from build123d import *

# Parameters (mm, degrees)
SKETCH_1_R      = 17.5
EXTRUDE_1_DEPTH = 57
SKETCH_2_R      = 23
EXTRUDE_2_DEPTH = 84
SKETCH_3_R      = 17
EXTRUDE_3_DEPTH = 6
SKETCH_4_R      = 13
EXTRUDE_4_DEPTH = 43
CHAMFER_1_SIZE  = 0.5


with BuildPart() as part:
    # 草图1 → 凸台-拉伸1 (new, symmetric)
    with BuildSketch(Plane.XY):
        with Locations(Location((0, 0, 0), (0, 0, 180))):
            Circle(SKETCH_1_R)
    extrude(amount=EXTRUDE_1_DEPTH, both=True)

    # 草图2 → 凸台-拉伸2 (add)
    with BuildSketch(Plane(origin=(0, 0, -57), x_dir=(-1, 0, 0), z_dir=(0, 0, -1))):
        with Locations(Location((0, 0, 0), (0, 0, 180))):
            Circle(SKETCH_2_R)
    extrude(amount=EXTRUDE_2_DEPTH)

    # 草图3 → 凸台-拉伸3 (add)
    with BuildSketch(Plane(origin=(0, 0, -141), x_dir=(-1, 0, 0), z_dir=(0, 0, -1))):
        Circle(SKETCH_3_R)
    extrude(amount=EXTRUDE_3_DEPTH)

    # 草图4 → 凸台-拉伸4 (add)
    with BuildSketch(Plane(origin=(0, 0, -147), x_dir=(-1, 0, 0), z_dir=(0, 0, -1))):
        Circle(SKETCH_4_R)
    extrude(amount=EXTRUDE_4_DEPTH)

    # 倒角1
    chamfer_1_edges = [part.edges().sort_by_distance(p)[0] for p in [
        (17, 0, -147),
        (13, 0, -190),
        (17.5, 0, 57),
        (-23, 0, -57),
        (-23, 0, -141),
    ]]
    chamfer(chamfer_1_edges, length=CHAMFER_1_SIZE)


solid = part.part
Build history of the part. All positions in model axes, mm. A direction names the side the tool comes from. Give positions to 0.01 mm unless a question says otherwise; leave off trailing zeros. Order: outer loops, then holes, each group sorted by start corner. A loop starts at its lowest first (then second) coordinate and runs counter-clockwise, first axis right, second up. Notation, with made-up numbers: M 68,-24 L 109,-24 A5 cw 109,-17 Z; hole C 4.5,31 d4. An arc over 180 degrees is marked long. Put each result on its own line as item: value.
Item 1: Cut at C-C on z = -18. Write the cut outline in (x, y).
Results are:
outline: C 0,0 d35
Item 2: Which spindle directions (+Z, -Z, +X, -X, +Y, -Y) get a long thin tool onto all of the face, cutting with end or side? Do faces 1 (the face through (3.794, 17.084, 0.544)), 2 (the face through (0, 0, -190)), 3 (the face through (10.316, -7.91, -167.952)). Say none if no direction does.
Results are:
face 1: +Z
face 2: -Z, +X, -X, +Y, -Y
face 3: -Z
Item 3: Cut at A-A on x = 0. Write the cut outline in (y, z).
Results are:
outline: M -23,-140.5 L -22.5,-141 L -17,-141 L -17,-146.5 L -16.5,-147 L -13,-147 L -13,-189.5 L -12.5,-190 L 12.5,-190 L 13,-189.5 L 13,-147 L 16.5,-147 L 17,-146.5 L 17,-141 L 22.5,-141 L 23,-140.5 L 23,-57.5 L 22.5,-57 L 17.5,-57 L 17.5,56.5 L 17,57 L -17,57 L -17.5,56.5 L -17.5,-57 L -22.5,-57 L -23,-57.5 Z
Item 4: Drop flat-ended pins along their axis: pin 1 Ø3 at (y, z) = (16, -18.5) entering from +X; pin 2 Ø8 at (x, y) = (-2.5, 17.5) entering from -Z; pin 3 Ø3 at (y, z) = (4.5, 29.5) entering from +X; pin 4 Ø4 at (x, y) = (18.5, 17) entering from -Z. Give the stop position or say it passes through.
Results are:
pin 1: x = 9.8
pin 2: z = -147
pin 3: x = 17.24
pin 4: through
Item 5: Wall check: probe 1 along Y at (x, z) = (1, -55.5); probe 2 along Z at (x, y) = (8, -11); probe 3 along Z at (x, y) = (19.5, -9). Give the ranges that are in metal, low to high.
Results are:
probe 1: -17.47 to 17.47
probe 2: -147 to 57
probe 3: -141 to -57
